```python
from build123d import *

# Parameters (mm, degrees)
SKETCH1_W           = 88
SKETCH1_H           = 27
BOSS_EXTRUDE1_DEPTH = 2
SKETCH2_R           = 1.6
CUT_EXTRUDE1_DEPTH  = 47.067884692
FILLET1_R           = 2
CUT_EXTRUDE2_DEPTH  = 47.067884692
M3_TAPPED_HOLE1_D   = 2.5
SKETCH6_R           = 1.6
CUT_EXTRUDE3_DEPTH  = 47.067884692


with BuildPart() as part:
    # Sketch1 → Boss-Extrude1 (new body)
    with BuildSketch(Plane(origin=(0, 0, 0), x_dir=(1, 0, 0), z_dir=(0, 1, 0))):
        Rectangle(SKETCH1_W, SKETCH1_H)
    extrude(amount=BOSS_EXTRUDE1_DEPTH)

    # Sketch2 → Cut-Extrude1 (cut, through all)
    with BuildSketch(Plane(origin=(0, 2, 0), x_dir=(1, 0, 0), z_dir=(0, 1, 0))):
        with Locations(Location((-40.5, 10, 0), (0, 0, 270))):
            Circle(SKETCH2_R)
        with Locations(Location((40.5, 10, 0), (0, 0, 270))):
            Circle(SKETCH2_R)
        with Locations(Location((40.5, -10, 0), (0, 0, 270))):
            Circle(SKETCH2_R)
        with Locations(Location((-40.5, -10, 0), (0, 0, 270))):
            Circle(SKETCH2_R)
    extrude(amount=-CUT_EXTRUDE1_DEPTH, mode=Mode.SUBTRACT)

    # Fillet1
    fillet1_edges = [part.edges().sort_by_distance(p)[0] for p in [
        (44, 1, 13.5),
        (-44, 1, 13.5),
        (-44, 1, -13.5),
        (44, 1, -13.5),
    ]]
    fillet(fillet1_edges, radius=FILLET1_R)

    # Sketch3 → Cut-Extrude2 (cut, through all)
    with BuildSketch(Plane(origin=(0, 2, 0), x_dir=(1, 0, 0), z_dir=(0, 1, 0))):
        with BuildLine():
            Line((-29.863538607, 3.233244374), (-28.576351648, -4.066755626))
            ThreePointArc((-28.576351648, -4.066755626), (-27.755503304, -5.488506663), (-26.212813041, -6.05))
            Line((-26.212813041, -6.05), (26.212813041, -6.05))
            ThreePointArc((26.212813041, -6.05), (27.755503304, -5.488506663), (28.576351648, -4.066755626))
            Line((28.576351648, -4.066755626), (29.863538607, 3.233244374))
            ThreePointArc((29.863538607, 3.233244374), (29.338506663, 5.192690263), (27.5, 6.05))
            Line((27.5, 6.05), (-27.5, 6.05))
            ThreePointArc((-27.5, 6.05), (-29.338506663, 5.192690263), (-29.863538607, 3.233244374))
        make_face()
    extrude(amount=-CUT_EXTRUDE2_DEPTH, mode=Mode.SUBTRACT)

    # M3 Tapped Hole1 (through all)
    with Locations(Plane(origin=(0, 2, 0), x_dir=(1, 0, 0), z_dir=(0, 1, 0))):
        with Locations((-31.75, 0), (31.75, 0)):
            Hole(M3_TAPPED_HOLE1_D / 2)

    # Sketch6 → Cut-Extrude3 (cut, through all)
    with BuildSketch(Plane(origin=(0, 2, 0), x_dir=(1, 0, 0), z_dir=(0, 1, 0))):
        with Locations(Location((-31.75, 0, 0), (0, 0, 270))):
            Circle(SKETCH6_R)
        with Locations(Location((31.75, 0, 0), (0, 0, 270))):
            Circle(SKETCH6_R)
    extrude(amount=-CUT_EXTRUDE3_DEPTH, mode=Mode.SUBTRACT)


solid = part.part
```
For this review, take the finished solid that the model builds, in its own axes (mm). A direction names the side the tool comes from. Coordinates: 2 decimals unless noted, no trailing zeros. Write each loop counter-clockwise with the first axis right and the second up, starting at its lowest first coordinate (ties: lowest second). Pieces come first, ordered by that corner, then holes. Notation, with made-up numbers: (75.25, 26.5) - (80.25, 26.5) arc R18 ccw to (80.25, 44.5) - close; hole circle Ø9 at (29.25, 22). An arc over 180 degrees is marked (long way). Answer in a Markdown table with one row per item. Add a question column.
Q1. We need section C-C, the plane y = 1.45. State the section outline as (x, z) points, and give its area (3 significant figures).
Q2. For probe 1 along X at (y, z) = (1, 10); probe 2 along X at (y, z) = (0.3, 0.25); probe 3 along Z at (x, y) = (-5.5, 0.45), list the stretches that pass through material, from the lowest coordinate up.
Q3. We need section D-D, the plane x = 40.5. State the section outline as (y, z) points.
Q4. For P1, Ø3, axis at x = -40.5, z = 10, coming from the -Y side; P2, Ø3.5, axis at x = -31.75, z = 0, coming from the -Y side, all flat-tipped, find the tip position at first contact; note any pin that passes through.
Q5. Draft analysis for pull direction Z (two halves, no side actions). For faces 3 (the flat face through (44, 1, 0)), 4 (the cylindrical face through (43.4, 1.01, -12.93)), 5 (the cylindrical face through (30.19, 1.01, -0.35)), state which applies: +Z half, -Z half, draft (parallel to the pull), parting line (faces both ways), or undercut.
Q6. We need section B-B, the plane x = -15. State the section outline as (y, z) points, and give its area (3 significant figures).
Q7. We need section A-A, the plane z = 10. State the section outline as (x, y) points.
Q8. Tool access review of faces 1 (the cylindrical face through (-43.43, 1.01, -12.9)), 2 (the flat face through (-29.23, 1.01, 0.37)): name each direction out of +Z, -Z, +X, -X, +Y, -Y from which nothing blocks a thin tool from reaching the whole face with its end or side.
Answer list:
| question | item | result |
|---|---|---|
| 1 | outline | (-44, -11.5) arc R2 ccw to (-42, -13.5) - (42, -13.5) arc R2 ccw to (44, -11.5) - (44, 11.5) arc R2 ccw to (42, 13.5) - (-42, 13.5) arc R2 ccw to (-44, 11.5) - close; hole circle Ø3.2 at (-40.5, -10); hole circle Ø3.2 at (-40.5, 10); hole circle Ø3.2 at (-31.75, 0); hole (-29.86, -3.23) arc R2.4 ccw to (-27.5, -6.05) - (27.5, -6.05) arc R2.4 ccw to (29.86, -3.23) - (28.58, 4.07) arc R2.4 ccw to (26.21, 6.05) - (-26.21, 6.05) arc R2.4 ccw to (-28.58, 4.07) - close; hole circle Ø3.2 at (31.75, 0); hole circle Ø3.2 at (40.5, -10); hole circle Ø3.2 at (40.5, 10) |
| 1 | area | 1,620 mm2 |
| 2 | probe 1 | x = -44 to -42.1, -38.9 to 38.9, 42.1 to 44 |
| 2 | probe 2 | x = -44 to -33.33, -30.17 to -29.25, 29.25 to 30.17, 33.33 to 44 |
| 2 | probe 3 | z = -13.5 to -6.05, 6.05 to 13.5 |
| 3 | outline | (0, -13.5) - (2, -13.5) - (2, -11.6) - (0, -11.6) - close; (0, -8.4) - (2, -8.4) - (2, 8.4) - (0, 8.4) - close; (0, 11.6) - (2, 11.6) - (2, 13.5) - (0, 13.5) - close |
| 4 | P1 | passes through |
| 4 | P2 | stops at y = 0 |
| 5 | face 3 | draft |
| 5 | face 4 | -Z half |
| 5 | face 5 | undercut |
| 6 | outline | (0, -13.5) - (2, -13.5) - (2, -6.05) - (0, -6.05) - close; (0, 6.05) - (2, 6.05) - (2, 13.5) - (0, 13.5) - close |
| 6 | area | 29.8 mm2 |
| 7 | outline | (-44, 0) - (-42.1, 0) - (-42.1, 2) - (-44, 2) - close; (-38.9, 0) - (38.9, 0) - (38.9, 2) - (-38.9, 2) - close; (42.1, 0) - (44, 0) - (44, 2) - (42.1, 2) - close |
| 8 | face 1 | -Z, -X, +Y, -Y |
| 8 | face 2 | +Y, -Y |
